Here's how the part is built. I have some questions about the finished solid (model axes, mm). Face numbers are marked on the shaded views. A direction names the side the tool comes from. Round coordinates to 2 decimals unless told otherwise and drop trailing zeros. Write each loop counter-clockwise with the first axis right and the second up, starting at its lowest first coordinate (ties: lowest second). Pieces come first, ordered by that corner, then holes. Notation, with made-up numbers: (-39.75, 41.25) -> (3.25, 41.25) arc R20 cw to (3.25, 75.25) -> close; hole circle Ø6 at (79.5, -26.75). An arc over 180 degrees is marked (long way). Put each result on its own line as item: value. Start each with the question number.
1) I want a section at B-B, the plane z = 83. List the corners of the cut face in (x, y) for me, then the cut area to 3 significant figures.
2) I want a section at C-C, the plane y = -257. List the corners of the cut face in (x, z) for me, then the cut area to 3 significant figures.
3) We'd pull the mould along Y, two halves only. Please class the marked faces 6, 7 and 8: released by +Y, released by -Y, zero draft, split by the parting line, or undercut.
4) If I drill on line 1 along Y through (x, z) = (38.5, 32); line 2 along Z through (x, y) = (43.5, -42.5); line 3 along Y through (x, z) = (-44, 139), over which ranges is the centre line in solid material (lowest first)? Write a range as [from, to].
5) Will these pins go through, and if not, where does the flat tip stop? P1, Ø11, axis at y = -333.5, z = 85, coming from the -X side; P2, Ø11, axis at y = -337, z = 98, coming from the +X side; P3, Ø11, axis at x = 19, y = -335, coming from the -Z side; P4, Ø6, axis at y = -146, z = 46, coming from the -X side.
6) I want a section at D-D, the plane x = 0. List the corners of the cut face in (y, z) for me, then the cut area to 3 significant figures.
7) I want a section at A-A, the plane x = 73. List the corners of the cut face in (y, z) for me.
8) Which directions (+Z, -Z, +X, -X, +Y, -Y) give clear straight access to the entire face, cutting with the end or side of a thin tool? Please do the marked faces 1, 2, 3, 4 and 5.
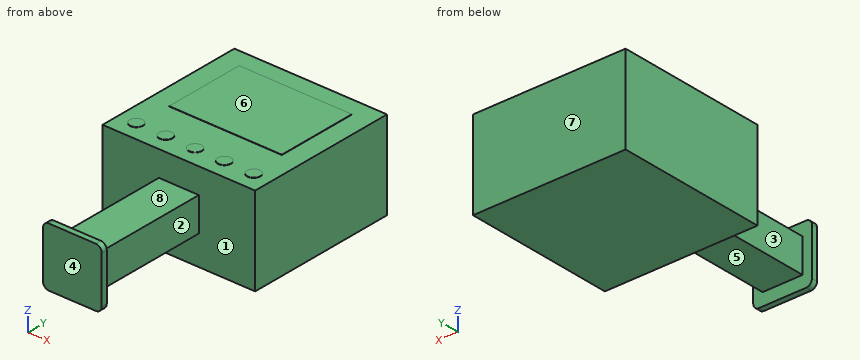
from build123d import *

# Parameters (mm, degrees)
SKETCH1_W           = 260
SKETCH1_H           = 260
BOSS_EXTRUDE1_DEPTH = 150
SKETCH2_R           = 11.25
SKETCH2_W           = 192
SKETCH2_H           = 138
BOSS_EXTRUDE2_DEPTH = 0.5
SKETCH3_W           = 68.073396254
SKETCH3_H           = 57.221115693
BOSS_EXTRUDE3_DEPTH = 200
SKETCH4_W           = 100
SKETCH4_H           = 100
BOSS_EXTRUDE4_DEPTH = 10
FILLET1_R           = 10


with BuildPart() as part:
    # Sketch1 → Boss-Extrude1 (new body)
    with BuildSketch(Plane.XY):
        Rectangle(SKETCH1_W, SKETCH1_H)
    extrude(amount=BOSS_EXTRUDE1_DEPTH)

    # Sketch2 → Boss-Extrude2 (add)
    with BuildSketch(Plane.XY.offset(150)):
        with Locations((-100, -98)):
            Circle(SKETCH2_R)
        with Locations((-50, -98)):
            Circle(SKETCH2_R)
        with Locations(Location((50, -98, 0), (0, 0, 180))):
            Circle(SKETCH2_R)
        with Locations(Location((100, -98, 0), (0, 0, 180))):
            Circle(SKETCH2_R)
        with Locations(Location((0, -98, 0), (0, 0, 180))):
            Circle(SKETCH2_R)
        with Locations((0, 31)):
            Rectangle(SKETCH2_W, SKETCH2_H)
    extrude(amount=BOSS_EXTRUDE2_DEPTH)

    # Sketch3 → Boss-Extrude3 (add)
    with BuildSketch(Plane.XZ.offset(130)):
        with Locations((0, 78.579676991)):
            Rectangle(SKETCH3_W, SKETCH3_H)
    extrude(amount=BOSS_EXTRUDE3_DEPTH)

    # Sketch4 → Boss-Extrude4 (add)
    with BuildSketch(Plane.XZ.offset(330)):
        with Locations((0, 78.579676991)):
            Rectangle(SKETCH4_W, SKETCH4_H)
    extrude(amount=BOSS_EXTRUDE4_DEPTH)

    # Fillet1
    fillet1_edges = [part.edges().sort_by_distance(p)[0] for p in [
        (50, -335, 28.579676991),
        (50, -335, 128.579676991),
        (-50, -335, 128.579676991),
        (-50, -335, 28.579676991),
    ]]
    fillet(fillet1_edges, radius=FILLET1_R)


solid = part.part
Findings:
1. outline: (-130, -130) -> (-34.04, -130) -> (-34.04, -330) -> (-50, -330) -> (-50, -340) -> (50, -340) -> (50, -330) -> (34.04, -330) -> (34.04, -130) -> (130, -130) -> (130, 130) -> (-130, 130) -> close
1. area: 82,200 mm2
2. outline: (-34.04, 49.97) -> (34.04, 49.97) -> (34.04, 107.19) -> (-34.04, 107.19) -> close
2. area: 3,900 mm2
3. face 6: zero draft
3. face 7: released by +Y
3. face 8: undercut
4. line 1: y = [-340, -330], [-130, 130]
4. line 2: z = [0, 150]
4. line 3: y = [-130, 130]
5. P1: stops at x = -50
5. P2: stops at x = 50
5. P3: stops at z = 28.58
5. P4: passes through
6. outline: (-340, 28.58) -> (-330, 28.58) -> (-330, 49.97) -> (-130, 49.97) -> (-130, 0) -> (130, 0) -> (130, 150) -> (100, 150) -> (100, 150.5) -> (-38, 150.5) -> (-38, 150) -> (-86.75, 150) -> (-86.75, 150.5) -> (-109.25, 150.5) -> (-109.25, 150) -> (-130, 150) -> (-130, 107.19) -> (-330, 107.19) -> (-330, 128.58) -> (-340, 128.58) -> close
6. area: 51,500 mm2
7. outline: (-130, 0) -> (130, 0) -> (130, 150) -> (100, 150) -> (100, 150.5) -> (-38, 150.5) -> (-38, 150) -> (-130, 150) -> close
8. face 1: none
8. face 2: +Z, -Z, +X
8. face 3: +Z, -Z, -X
8. face 4: +Z, -Z, +X, -X, -Y
8. face 5: -Z, +X, -X
